from build123d import *

# Parameters (mm, degrees)
SKETCH_1_R               = 450
SKETCH_1_R_2             = 42.5
EXTRUDE_1_DEPTH          = 20
PATTERN_CIRCULAR_1_COUNT = 24
SKETCH_7_R               = 125
SKETCH_7_R_2             = 42.5
EXTRUDE_2_DEPTH          = 30
SKETCH_8_R               = 175
SKETCH_8_R_2             = 42.5
EXTRUDE_3_DEPTH          = 20
SKETCH_9_R               = 90
CUT_EXTRUDE_1_DEPTH      = 34


with BuildPart() as part:
    # 草图1 → 凸台-拉伸1 (new, symmetric)
    with BuildSketch(Plane.XY):
        Circle(SKETCH_1_R)
        Circle(SKETCH_1_R_2, mode=Mode.SUBTRACT)
    extrude(amount=EXTRUDE_1_DEPTH, both=True)

    # 草图4 → M42 六角头螺栓的柱形沉头孔1 (revolve, cut)
    with BuildSketch(Plane(origin=(0, 410, 20), x_dir=(0, -1, 0), z_dir=(1, 0, 0))):
        Polygon((0, 0), (0, 62.017212381), (20, 50), (20, 20), (30, 20), (30, 0), align=None)
    hole_wizard_m42_1 = revolve(axis=Axis((0, 410, 26.35), (0, 0, -1)), mode=Mode.SUBTRACT)

    # 阵列(圆周)1: M42 六角头螺栓的柱形沉头孔1 ×24 about axis
    pattern_circular_1_axis = Axis((0, 0, 0), (0, 0, 1))
    for i in range(1, PATTERN_CIRCULAR_1_COUNT):
        add(hole_wizard_m42_1.rotate(pattern_circular_1_axis, i * 360 / PATTERN_CIRCULAR_1_COUNT), mode=Mode.SUBTRACT)

    # 草图7 → 凸台-拉伸2 (add)
    with BuildSketch(Plane.XY.offset(20)):
        Circle(SKETCH_7_R)
        Circle(SKETCH_7_R_2, mode=Mode.SUBTRACT)
    extrude(amount=EXTRUDE_2_DEPTH)

    # 草图8 → 凸台-拉伸3 (add)
    with BuildSketch(Plane.XY.offset(50)):
        Circle(SKETCH_8_R)
        Circle(SKETCH_8_R_2, mode=Mode.SUBTRACT)
    extrude(amount=EXTRUDE_3_DEPTH)

    # 草图9 → 切除-拉伸1 (cut)
    with BuildSketch(Plane(origin=(0, 0, -20), x_dir=(-1, 0, 0), z_dir=(0, 0, -1))):
        Circle(SKETCH_9_R)
    extrude(amount=-CUT_EXTRUDE_1_DEPTH, mode=Mode.SUBTRACT)


solid = part.part
Geometry: final body of the model. Coordinates: model frame, mm. A direction names the side the tool comes from. Coordinates: 2 decimals unless noted, no trailing zeros. Order: outer loops, then holes, each group sorted by start corner. A loop starts at its lowest first (then second) coordinate and runs counter-clockwise, first axis right, second up.
(1) Section query B-B (z = 38). Return the cut outline in (x, y), plus the area to 3 significant figures.
(2) Material intervals for probe 1 along Y at (x, z) = (0, -6.5); probe 2 along Y at (x, z) = (-337, -3); probe 3 along X at (y, z) = (-285.5, 13), sorted ascending.
(3) Draft query along X for faces 1 (the face through (-124.88, 5.5, 34.79)), 2 (the face through (36, -36, 70)), 3 (the face through (397, -127, 0)), 4 (the face through (190.26, 341.55, -9.86)). Return one class per face: pulls with the +X half, pulls with the -X half, needs draft (parallel to the pull), parting line crosses it, or undercut.
(4) First-contact query: pin 1 (8 mm diameter, centred on x = 128.5, z = 50, fed in from +Y); pin 2 (4 mm diameter, centred on x = -325, y = -223, fed in from +Z); pin 3 (10 mm diameter, centred on x = 99, z = 28, fed in from +Y). Flat tips, straight axial feed; report the tip coordinate or a pass-through.
(5) Section query A-A (x = 0). State how many separate pieces and enclosed holes the cut face has, plus the area to 3 significant figures.
(6) Access query for faces 5 (the face through (-397, 127, 0)), 6 (the face through (-391.525, 7.66, -9.86)). Directions: +Z, -Z, +X, -X, +Y, -Y. A direction counts if a zero-diameter tool reaches every point of the face in a straight line with its end or side. Return the directions, or none.
Solution:
1. outline: circle Ø250 at (0, 0); hole circle Ø85 at (0, 0)
1. area: 43,400 mm2
2. probe 1: y = -450 to -430, -390 to -90, 90 to 390, 430 to 450
2. probe 2: y = -298.21 to -213.57, -196.43 to 196.43, 213.57 to 298.21
2. probe 3: x = -347.84 to -319.59, -260.24 to 260.24, 319.59 to 347.84
3. face 1: parting line crosses it
3. face 2: needs draft
3. face 3: undercut
3. face 4: undercut
4. pin 1: stops at y = 122.98
4. pin 2: stops at z = 20
4. pin 3: stops at y = 82.4
5. separate pieces: 4
5. enclosed holes: 0
5. area: 35,600 mm2
6. face 5: +Z
6. face 6: +Z, -Z
